from build123d import *

# Parameters (mm, degrees)
SKETCH1_W           = 60
SKETCH1_H           = 62
BOSS_EXTRUDE1_DEPTH = 8
SKETCH3_R           = 19.25
CUT_EXTRUDE1_DEPTH  = 2
SKETCH4_R           = 5
CUT_EXTRUDE2_DEPTH  = 44.554563481


with BuildPart() as part:
    # Sketch1 → Boss-Extrude1 (new body)
    with BuildSketch(Plane.XY):
        Rectangle(SKETCH1_W, SKETCH1_H)
    extrude(amount=BOSS_EXTRUDE1_DEPTH)

    # Sketch3 → Cut-Extrude1 (cut)
    with BuildSketch(Plane.XY.offset(8)):
        Circle(SKETCH3_R)
    extrude(amount=-CUT_EXTRUDE1_DEPTH, mode=Mode.SUBTRACT)

    # Sketch4 → Cut-Extrude2 (cut, through all)
    with BuildSketch(Plane.XY.offset(6)):
        Circle(SKETCH4_R)
    extrude(amount=-CUT_EXTRUDE2_DEPTH, mode=Mode.SUBTRACT)


solid = part.part
Build history of the part. All positions in model axes, mm. A direction names the side the tool comes from. Coordinates: 2 decimals unless noted, no trailing zeros. Order: outer loops, then holes, each group sorted by start corner. A loop starts at its lowest first (then second) coordinate and runs counter-clockwise, first axis right, second up. Notation, with made-up numbers: (-27, 8.25) - (0, 8.25) arc R16 ccw to (0, 20.25) - close; hole circle Ø3 at (76.25, -36). An arc over 180 degrees is marked (long way). Write each question's results on one line, items separated by ' | '. Start each with the question number.
Item 1: Band-saw the part on D-D on x = 7. Write the cut outline in (y, z).
Item 2: Mould opens along Y. For faces 3 (the face through (0, -31, 4)), 4 (the face through (-1.08, -4.88, 3.04)), 5 (the face through (-30, 0, 4)), 6 (the face through (4, -4, 6)) say: released by +Y, released by -Y, zero draft, split by the parting line, or undercut.
Item 3: Tool access for faces 1 (the face through (-14, 14, 8)), 2 (the face through (-15.28, -11.71, 7.01)): list every direction of +Z, -Z, +X, -X, +Y, -Y with a clear straight run to the whole face (end or side of a thin tool).
Item 4: Flat gauge pin, fed straight in: pin 1 (9 mm diameter, centred on x = 0, y = 0, fed in from -Z). Where does the tip first touch, or does it go through?
Item 5: Wall check: probe 1 along Y at (x, z) = (0, 6.5); probe 2 along Z at (x, y) = (-11, -2.5); probe 3 along X at (y, z) = (1.5, 6.75). Give the ranges that are in metal, low to high. Write a range as [from, to].
Item 6: Band-saw the part on C-C on z = 1. Write the cut outline in (x, y), and give its area (3 significant figures).
Item 7: Band-saw the part on B-B on y = 0. Write the cut outline in (x, z).
Item 8: Band-saw the part on A-A on x = 0. Write the cut outline in (y, z), and give its area (3 significant figures).
Numbers:
1) outline: (-31, 0) - (31, 0) - (31, 8) - (17.93, 8) - (17.93, 6) - (-17.93, 6) - (-17.93, 8) - (-31, 8) - close
2) face 3: released by -Y | face 4: undercut | face 5: zero draft | face 6: undercut
3) face 1: +Z, +X, -X, +Y, -Y | face 2: +Z
4) pin 1: through
5) probe 1: [-31, -19.25], [19.25, 31] | probe 2: [0, 6] | probe 3: [-30, -19.19], [19.19, 30]
6) outline: (-30, -31) - (30, -31) - (30, 31) - (-30, 31) - close; hole circle Ø10 at (0, 0) | area: 3,640 mm^2
7) outline: (-30, 0) - (-5, 0) - (-5, 6) - (-19.25, 6) - (-19.25, 8) - (-30, 8) - close; (5, 0) - (30, 0) - (30, 8) - (19.25, 8) - (19.25, 6) - (5, 6) - close
8) outline: (-31, 0) - (-5, 0) - (-5, 6) - (-19.25, 6) - (-19.25, 8) - (-31, 8) - close; (5, 0) - (31, 0) - (31, 8) - (19.25, 8) - (19.25, 6) - (5, 6) - close | area: 359 mm^2
